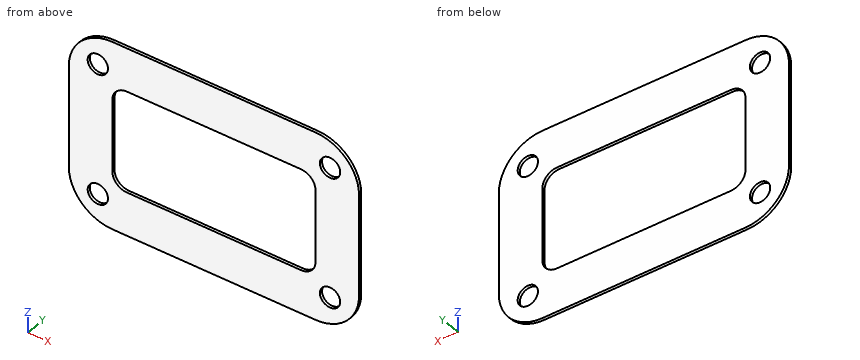
```python
from build123d import *

# Parameters (mm, degrees)
BOSS_EXTRUDE1_DEPTH  = 1
CUT_EXTRUDE1_DEPTH   = 60.642686056
HOLE1_D              = 7
LPATTERN1_COUNT      = 2
LPATTERN1_PITCH      = 80
LPATTERN1_COUNT_DIR2 = 2
LPATTERN1_PITCH_DIR2 = 45


with BuildPart() as part:
    # Sketch1 → Boss-Extrude1 (new body)
    with BuildSketch(Plane(origin=(0, 0, 0), x_dir=(1, 0, 0), z_dir=(0, 1, 0))):
        with BuildLine():
            Line((-35, 32.5), (35, 32.5))
            ThreePointArc((35, 32.5), (45.606601718, 28.106601718), (50, 17.5))
            Line((50, 17.5), (50, -17.5))
            ThreePointArc((50, -17.5), (45.606601718, -28.106601718), (35, -32.5))
            Line((35, -32.5), (-35, -32.5))
            ThreePointArc((-35, -32.5), (-45.606601718, -28.106601718), (-50, -17.5))
            Line((-50, -17.5), (-50, 17.5))
            ThreePointArc((-50, 17.5), (-45.606601718, 28.106601718), (-35, 32.5))
        make_face()
    extrude(amount=BOSS_EXTRUDE1_DEPTH)

    # Sketch2 → Cut-Extrude1 (cut, through all)
    with BuildSketch(Plane(origin=(0, 1, 0), x_dir=(1, 0, 0), z_dir=(0, 1, 0))):
        with BuildLine():
            Line((-30, 17.5), (30, 17.5))
            ThreePointArc((30, 17.5), (33.535533906, 16.035533906), (35, 12.5))
            Line((35, 12.5), (35, -12.5))
            ThreePointArc((35, -12.5), (33.535533906, -16.035533906), (30, -17.5))
            Line((30, -17.5), (-30, -17.5))
            ThreePointArc((-30, -17.5), (-33.535533906, -16.035533906), (-35, -12.5))
            Line((-35, -12.5), (-35, 12.5))
            ThreePointArc((-35, 12.5), (-33.535533906, 16.035533906), (-30, 17.5))
        make_face()
    extrude(amount=-CUT_EXTRUDE1_DEPTH, mode=Mode.SUBTRACT)

    # Hole1 (through all)
    with Locations(Plane(origin=(-40, 1, -22.5), x_dir=(0, 0, 1), z_dir=(0, 1, 0))):
        with Locations((0, 0)):
            hole1 = Hole(HOLE1_D / 2)

    # LPattern1: Hole1 2 × 2
    with Locations(*[(i * LPATTERN1_PITCH, 0, j * LPATTERN1_PITCH_DIR2) for i in range(LPATTERN1_COUNT) for j in range(LPATTERN1_COUNT_DIR2) if (i, j) != (0, 0)]):
        add(hole1, mode=Mode.SUBTRACT)


solid = part.part
```
Can you work these out from the model? Positions are in its coordinate system, mm. Give positions to 0.01 mm unless a question says otherwise; leave off trailing zeros. Loops run counter-clockwise (first coordinate to the right, second up) from the corner with the lowest first, then second, coordinate; pieces in that order, holes last. Notation, with made-up numbers: M 72.5,19 L 105.5,19 A15 cw 105.5,37 Z; hole C -32,75.5 d10. An arc over 180 degrees is marked long. Answer in a Markdown table with one row per item.
1. Suppose I cut it at B-B on z = 0. Write out the boundary of the cut face in (x, y).
Taken from the geometry:
| item | result |
|---|---|
| outline | M -50,0 L -35,0 L -35,1 L -50,1 Z; M 35,0 L 50,0 L 50,1 L 35,1 Z |
2. Suppose I cut it at C-C on y = 0.6. Write out the boundary of the cut face in (x, z), plus the area to 3 significant figures.
Taken from the geometry:
| item | result |
|---|---|
| outline | M -50,-17.5 A15 ccw -35,-32.5 L 35,-32.5 A15 ccw 50,-17.5 L 50,17.5 A15 ccw 35,32.5 L -35,32.5 A15 ccw -50,17.5 Z; hole C -40,-22.5 d7; hole C -40,22.5 d7; hole M -35,-12.5 A5 ccw -30,-17.5 L 30,-17.5 A5 ccw 35,-12.5 L 35,12.5 A5 ccw 30,17.5 L -30,17.5 A5 ccw -35,12.5 Z; hole C 40,-22.5 d7; hole C 40,22.5 d7 |
| area | 3,720 mm² |
3. If I drill on line 1 along Z through (x, y) = (25, 0.2); line 2 along X through (y, z) = (0.2, 2); line 3 along X through (y, z) = (0.55, 22.5), over which ranges is the centre line in solid material (lowest first)?
Taken from the geometry:
| item | result |
|---|---|
| line 1 | z = -32.5 to -17.5, 17.5 to 32.5 |
| line 2 | x = -50 to -35, 35 to 50 |
| line 3 | x = -49.14 to -43.5, -36.5 to 36.5, 43.5 to 49.14 |
4. Suppose I cut it at D-D on z = -21.5. Write out the boundary of the cut face in (x, y), plus the area to 3 significant figures.
Taken from the geometry:
| item | result |
|---|---|
| outline | M -49.46,0 L -43.35,0 L -43.35,1 L -49.46,1 Z; M -36.65,0 L 36.65,0 L 36.65,1 L -36.65,1 Z; M 43.35,0 L 49.46,0 L 49.46,1 L 43.35,1 Z |
| area | 85.5 mm² |
5. Suppose I cut it at A-A on x = -34. Write out the boundary of the cut face in (y, z), plus the area to 3 significant figures.
Taken from the geometry:
| item | result |
|---|---|
| outline | M 0,-32.5 L 1,-32.5 L 1,-15.5 L 0,-15.5 Z; M 0,15.5 L 1,15.5 L 1,32.5 L 0,32.5 Z |
| area | 34.0 mm² |
